from build123d import *

# Parameters (mm, degrees)
SKETCH_1_R               = 12.5
EXTRUDE_1_DEPTH          = 280
SKETCH_2_R               = 10
EXTRUDE_2_DEPTH          = 12
EXTRUDE_START            = 12
SKETCH_3_R               = 10
EXTRUDE_3_DEPTH          = 12
SKETCH_4_R               = 7.5
EXTRUDE_4_DEPTH          = 25
SKETCH_5_R               = 1.5
CUT_EXTRUDE_1_DEPTH      = 280
PATTERN_CIRCULAR_1_COUNT = 4


with BuildPart() as part:
    # 草图1 → 凸台-拉伸1 (new body)
    with BuildSketch(Plane.XY):
        Circle(SKETCH_1_R)
    extrude(amount=EXTRUDE_1_DEPTH)

    # 草图2 → 凸台-拉伸2 (add)
    with BuildSketch(Plane.XY.offset(280)):
        Circle(SKETCH_2_R)
    extrude(amount=EXTRUDE_2_DEPTH)

    # 草图3 → 凸台-拉伸3 (add)
    with BuildSketch(Plane(origin=(0, 0, 0), x_dir=(-1, 0, 0), z_dir=(0, 0, -1)).offset(EXTRUDE_START)):
        with Locations(Location((0, 0, 0), (0, 0, 180))):
            Circle(SKETCH_3_R)
    extrude(amount=-EXTRUDE_3_DEPTH)

    # 草图4 → 凸台-拉伸4 (add)
    with BuildSketch(Plane(origin=(0, 0, -12), x_dir=(-1, 0, 0), z_dir=(0, 0, -1))):
        Circle(SKETCH_4_R)
    extrude(amount=EXTRUDE_4_DEPTH)

    # 草图5 → 切除-拉伸1 (cut)
    with BuildSketch(Plane(origin=(0, 0, 0), x_dir=(-1, 0, 0), z_dir=(0, 0, -1))):
        with Locations((0, 13)):
            Circle(SKETCH_5_R)
    cut_extrude_1 = extrude(amount=-CUT_EXTRUDE_1_DEPTH, mode=Mode.SUBTRACT)

    # 阵列(圆周)1: 切除-拉伸1 ×4 about axis
    pattern_circular_1_axis = Axis((0, 0, 0), (0, 0, 1))
    for i in range(1, PATTERN_CIRCULAR_1_COUNT):
        add(cut_extrude_1.rotate(pattern_circular_1_axis, i * 360 / PATTERN_CIRCULAR_1_COUNT), mode=Mode.SUBTRACT)


solid = part.part
Can you work these out from the model? Positions are in its coordinate system, mm. A direction names the side the tool comes from. Round coordinates to 2 decimals unless told otherwise and drop trailing zeros. Loops run counter-clockwise (first coordinate to the right, second up) from the corner with the lowest first, then second, coordinate; pieces in that order, holes last. Notation, with made-up numbers: (73, 75.25) - (77, 75.25) arc R23 cw to (77, 103.25) - close; hole circle Ø9 at (65.25, 1). An arc over 180 degrees is marked (long way). Use CSV: the item, a comma, the result in double quotes. Start each with the question number.
1) If we section it at B-B on y = 4.5: Write out the boundary of the cut face in (x, z), plus the area to 3 significant figures.
2) For faces 1 (the cylindrical face through (8.922, 8.755, 138.04)), 2 (the flat face through (2, -10, 280)), 3 (the cylindrical face through (7.493, 0.33, -24.325)), which set-ups out of +Z, -Z, +X, -X, +Y, -Y let a thin tool reach every point of the face, with its end or its side?
3) Please list where these lines run through material, in increasing order: probe 1 along X at (y, z) = (4.75, 67); probe 2 along Z at (x, y) = (-8.5, -7); probe 3 along X at (y, z) = (7.5, 256.5). Write a range as [from, to].
4) If we section it at A-A on z = 205.5: Write out the boundary of the cut face in (x, y), plus the area to 3 significant figures.
5) For pin 1 Ø1 at (y, z) = (6.5, 209.5) entering from -X; pin 2 Ø1 at (x, y) = (6, 8) entering from -Z; pin 3 Ø12 at (y, z) = (7.5, 98) entering from +X, each with a flat end and sliding along its axis, tell me the tip position at first contact or that it passes through.
Geometry results:
1,outline,"(-11.66, 0) - (-8.93, 0) - (-8.93, -12) - (-6, -12) - (-6, -37) - (6, -37) - (6, -12) - (8.93, -12) - (8.93, 0) - (11.66, 0) - (11.66, 280) - (8.93, 280) - (8.93, 292) - (-8.93, 292) - (-8.93, 280) - (-11.66, 280) - close"
1,area,"7,260 mm2"
2,face 1,"+Z, -Z, +X, +Y"
2,face 2,"+Z"
2,face 3,"-Z"
3,probe 1,"x = [-11.56, 11.56]"
3,probe 2,"z = [0, 280]"
3,probe 3,"x = [-10, 10]"
4,outline,"(-12.42, -1.38) arc R12.5 ccw to (-1.38, -12.42) arc R1.5 cw to (1.38, -12.42) arc R12.5 ccw to (12.42, -1.38) arc R1.5 cw to (12.42, 1.38) arc R12.5 ccw to (1.38, 12.42) arc R1.5 cw to (-1.38, 12.42) arc R12.5 ccw to (-12.42, 1.38) arc R1.5 cw to start"
4,area,"483 mm2"
5,pin 1,"stops at x = -10.97"
5,pin 2,"stops at z = -12"
5,pin 3,"stops at x = 12.41"
